Here's how the part is built. I have some questions about the finished solid (model axes, mm). A direction names the side the tool comes from. Coordinates: 2 decimals unless noted, no trailing zeros. Write each loop counter-clockwise with the first axis right and the second up, starting at its lowest first coordinate (ties: lowest second). Pieces come first, ordered by that corner, then holes.
from build123d import *

# Parameters (mm, degrees)
BOSS_EXTRUDE1_DEPTH        = 10
SKETCH2_R                  = 14
CUT_EXTRUDE1_DEPTH         = 78.820305833
F_5_5_5_5_DIAMETER_HOLE1_D = 5.5
M3_TAPPED_HOLE1_D          = 2.5
FILLET1_R                  = 5
CHAMFER1_SIZE              = 0.5


with BuildPart() as part:
    # Sketch1 → Boss-Extrude1 (new body)
    with BuildSketch(Plane(origin=(0, 0, 0), x_dir=(0, 0, -1), z_dir=(1, 0, 0))):
        Polygon((0, -40), (0, 40), (10, 40), (10, 17.5), (66, 17.5), (66, -17.5), (10, -17.5), (10, -40), align=None)
    extrude(amount=BOSS_EXTRUDE1_DEPTH)

    # Sketch2 → Cut-Extrude1 (cut, through all)
    with BuildSketch(Plane(origin=(10, 0, 0), x_dir=(0, 0, -1), z_dir=(1, 0, 0))):
        with Locations((48, 0)):
            Circle(SKETCH2_R)
    extrude(amount=-CUT_EXTRUDE1_DEPTH, mode=Mode.SUBTRACT)

    # Ø5.5 (5.5) Diameter Hole1 (through all)
    with Locations(Plane.XY):
        with Locations((5, 32), (5, -32)):
            Hole(F_5_5_5_5_DIAMETER_HOLE1_D / 2)

    # M3 Tapped Hole1 (through all)
    with Locations(Plane(origin=(10, 0, 0), x_dir=(0, 0, -1), z_dir=(1, 0, 0))):
        with Locations((35.625631329, 12.374368671), (60.374368671, 12.374368671), (60.374368671, -12.374368671), (35.625631329, -12.374368671)):
            Hole(M3_TAPPED_HOLE1_D / 2)

    # Fillet1
    fillet1_edges = [part.edges().sort_by_distance(p)[0] for p in [
        (5, 17.5, -10),
        (5, -17.5, -10),
    ]]
    fillet(fillet1_edges, radius=FILLET1_R)

    # Chamfer1
    chamfer1_edges = [part.edges().sort_by_distance(p)[0] for p in [
        (0, 0, -34),
        (10, 0, -34),
    ]]
    chamfer(chamfer1_edges, length=CHAMFER1_SIZE)


solid = part.part
1. If I drill on line 1 (Y direction, x = 5, z = -2.75); line 2 (Y direction, x = 6.25, z = -3.5); line 3 (Y direction, x = 4.75, z = -36), over which ranges is the centre line in solid material (lowest first)?
2. I want a section at D-D (y = 32). List the corners of the cut face in (x, z) for me, then the cut area to 3 significant figures.
3. For pin 1 Ø2 at (y, z) = (-12.37, -60.37) entering from -X; pin 2 Ø6 at (x, y) = (6, -22.5) entering from -Z; pin 3 Ø3 at (x, y) = (5.5, 29.5) entering from -Z; pin 4 Ø2 at (x, z) = (6.5, -50.5) entering from -Y, each with a flat end and sliding along its axis, tell me the tip position at first contact or that it passes through.
4. I want a section at B-B (x = 3.5). List the corners of the cut face in (y, z) for me.
5. Thinking about a two-plate mould opening in Z: for faces 3 (the face through (5, 17.5, -40)), 4 (the face through (4.93, 12.429, -36.874)), 5 (the face through (4, 29, -10)), which applies, pulls with the +Z half, pulls with the -Z half, needs draft (parallel to the pull), parting line crosses it, or undercut?
6. On a 3-axis mill with a long thin cutter (end or side, diameter ignored), from which of +Z, -Z, +X, -X, +Y, -Y can I reach the whole of each face in a straight line? I mean faces 1 (the face through (5, -29, -10)), 2 (the face through (5.358, -29.273, -5.07)). Say none if no direction works.
7. I want a section at C-C (z = -4). List the corners of the cut face in (x, y) for me, then the cut area to 3 significant figures.
8. I want a section at A-A (y = 0). List the corners of the cut face in (x, z) for me, then the cut area to 4 significant figures.
Response values:
1. line 1: y = -40 to -34.75, -29.25 to 29.25, 34.75 to 40
1. line 2: y = -40 to -34.45, -29.55 to 29.55, 34.45 to 40
1. line 3: y = -17.5 to -13.57, -11.18 to -7.21, 7.21 to 11.18, 13.57 to 17.5
2. outline: (0, -10) - (2.25, -10) - (2.25, 0) - (0, 0) - close; (7.75, -10) - (10, -10) - (10, 0) - (7.75, 0) - close
2. area: 45.0 mm2
3. pin 1: passes through
3. pin 2: stops at z = -11
3. pin 3: stops at z = -10
3. pin 4: stops at y = -17.5
4. outline: (-40, -10) - (-34.3, -10) - (-34.3, 0) - (-40, 0) - close; (-29.7, -10) - (-22.5, -10) arc R5 cw to (-17.5, -15) - (-17.5, -66) - (17.5, -66) - (17.5, -15) arc R5 cw to (22.5, -10) - (29.7, -10) - (29.7, 0) - (-29.7, 0) - close; (34.3, -10) - (40, -10) - (40, 0) - (34.3, 0) - close; hole circle Ø28 at (0, -48); hole circle Ø2.5 at (-12.37, -60.37); hole circle Ø2.5 at (-12.37, -35.63); hole circle Ø2.5 at (12.37, -60.37); hole circle Ø2.5 at (12.37, -35.63)
5. face 3: needs draft
5. face 4: undercut
5. face 5: pulls with the -Z half
6. face 1: -Z, +X, -X, -Y
6. face 2: +Z, -Z
7. outline: (0, -40) - (10, -40) - (10, 40) - (0, 40) - close; hole circle Ø5.5 at (5, -32); hole circle Ø5.5 at (5, 32)
7. area: 752 mm2
8. outline: (0, -66) - (10, -66) - (10, -62.5) - (9.5, -62) - (0.5, -62) - (0, -62.5) - close; (0, -33.5) - (0.5, -34) - (9.5, -34) - (10, -33.5) - (10, 0) - (0, 0) - close
8. area: 379.5 mm2
